```python
from build123d import *

# Parameters (mm, degrees)
SKETCH1_W           = 850
SKETCH1_H           = 180
BOSS_EXTRUDE1_DEPTH = 20
CHAMFER1_SIZE       = 15


with BuildPart() as part:
    # Sketch1 → Boss-Extrude1 (new, symmetric)
    with BuildSketch(Plane.XY):
        Rectangle(SKETCH1_W, SKETCH1_H)
    extrude(amount=BOSS_EXTRUDE1_DEPTH, both=True)

    # Chamfer1
    chamfer1_edges = [part.edges().sort_by_distance(p)[0] for p in [
        (425, 0, 20),
        (-425, 0, 20),
        (0, 90, -20),
        (425, 0, -20),
        (0, -90, -20),
        (-425, 0, -20),
    ]]
    chamfer(chamfer1_edges, length=CHAMFER1_SIZE)


solid = part.part
```
The listing builds one solid part. Answer for the finished solid, in the listing's coordinates (mm). Coordinates: 2 decimals unless noted, no trailing zeros. Write each loop counter-clockwise with the first axis right and the second up, starting at its lowest first coordinate (ties: lowest second). Pieces come first, ordered by that corner, then holes.
Q1. Find the intervals of material crossed by line 1 along X through (y, z) = (10.5, -6); line 2 along Z through (x, y) = (-108.5, 76); line 3 along Y through (x, z) = (-42, -18), in increasing order.
Returned:
line 1: x = -424 to 424
line 2: z = -19 to 20
line 3: y = -77 to 77
Q2. Section B-B, the plane z = -12.5 is taken. Write down the section's boundary in (x, y).
Returned:
outline: (-417.5, -82.5) - (417.5, -82.5) - (417.5, 82.5) - (-417.5, 82.5) - close
Q3. Section A-A, the plane x = -310.5 is taken. Write down the section's boundary in (y, z).
Returned:
outline: (-90, -5) - (-75, -20) - (75, -20) - (90, -5) - (90, 20) - (-90, 20) - close
Q4. Given P1, Ø10, axis at y = -20.5, z = 15, coming from the +X side; P2, Ø12, axis at x = -217.5, z = -15.5, coming from the -Y side, each flat-ended and moving along its own axis, determine where each tip first touches the part or whether it passes through.
Returned:
P1: stops at x = 420
P2: stops at y = -85.5
